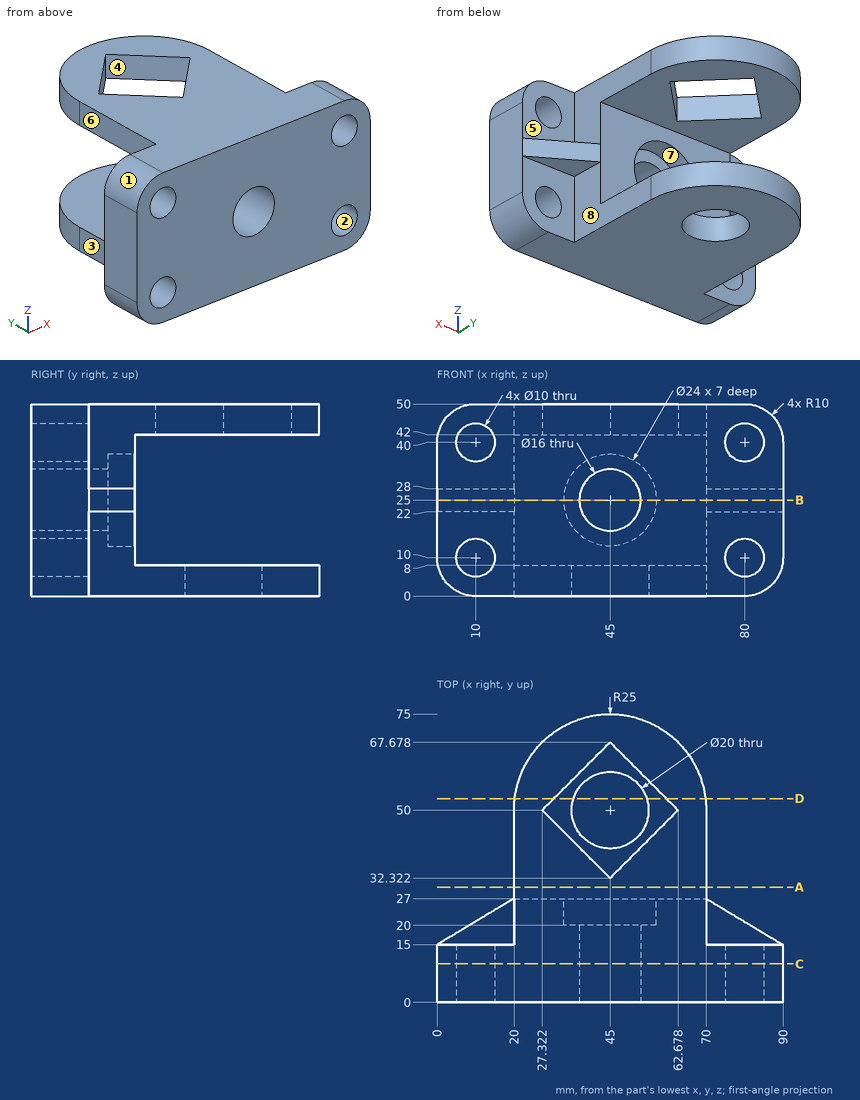
For this review, use the dimensioned drawing (mm, ordinates from the lowest corner) and the shaded views. A direction names the side the tool comes from. Coordinates: 2 decimals unless noted, no trailing zeros. Order: outer loops, then holes, each group sorted by start corner. A loop starts at its lowest first (then second) coordinate and runs counter-clockwise, first axis right, second up. Notation, with made-up numbers: (41.25, 64) - (73.25, 64) arc R18 cw to (73.25, 85) - close; hole circle Ø7 at (61, 38.25). An arc over 180 degrees is marked (long way). Use one line per item in the form item = value.
Q1. Draft analysis for pull direction Z (two halves, no side actions). For the marked faces 1, 2 and 3, state which applies: +Z half, -Z half, draft (parallel to the pull), parting line (faces both ways), or undercut.
Checked values:
face_1 = +Z half
face_2 = undercut
face_3 = draft
Q2. For probe 1 along X at (y, z) = (4, 40); probe 2 along Z at (x, y) = (8, 9); probe 3 along X at (y, z) = (6.75, 25), list the stretches that pass through material, from the lowest coordinate up. Write a range as from..to.
Checked values:
probe_1 = 0..5, 15..75, 85..90
probe_2 = 0.2..5.42, 14.58..35.42, 44.58..49.8
probe_3 = 0..37, 53..90
Q3. Consider section D-D (y = 53). Give the boundary of the cut face in (x, z).
Checked values:
outline = (20.18, 0) - (35.46, 0) - (35.46, 8) - (20.18, 8) - close; (20.18, 42) - (30.32, 42) - (30.32, 50) - (20.18, 50) - close; (54.54, 0) - (69.82, 0) - (69.82, 8) - (54.54, 8) - close; (59.68, 42) - (69.82, 42) - (69.82, 50) - (59.68, 50) - close
Q4. Consider section B-B (z = 25). Give the boundary of the cut face in (x, y).
Checked values:
outline = (0, 0) - (37, 0) - (37, 20) - (33, 20) - (33, 27) - (20, 27) - (0, 15) - close; (53, 0) - (90, 0) - (90, 15) - (70, 27) - (57, 27) - (57, 20) - (53, 20) - close
Q5. Consider section C-C (y = 10). Give the boundary of the cut face in (x, z).
Checked values:
outline = (0, 10) arc R10 ccw to (10, 0) - (80, 0) arc R10 ccw to (90, 10) - (90, 40) arc R10 ccw to (80, 50) - (10, 50) arc R10 ccw to (0, 40) - close; hole circle Ø10 at (10, 10); hole circle Ø10 at (10, 40); hole circle Ø16 at (45, 25); hole circle Ø10 at (80, 10); hole circle Ø10 at (80, 40)
Q6. For P1, Ø11, axis at y = 29.5, z = 15.5, coming from the +X side; P2, Ø6, axis at x = 76, z = 35, coming from the +Y side; P3, Ø12, axis at y = 37, z = 6.5, coming from the -X side, all flat-tipped, find the tip position at first contact; note any pin that passes through.
Checked values:
P1 = 70
P2 = 15
P3 = 20
Q7. Consider section A-A (y = 30). Give the boundary of the cut face in (x, z), then the cut area to 3 significant figures.
Checked values:
outline = (20, 0) - (70, 0) - (70, 8) - (20, 8) - close; (20, 42) - (70, 42) - (70, 50) - (20, 50) - close
area = 800 mm2
Q8. For the marked faces 4, 5, 6, 7 and 8, list the 3-axis set-ups (+Z, -Z, +X, -X, +Y, -Y) from which the entire face can be reached by the end or side of a thin tool; tool diameter is ignored.
Checked values:
face_4 = +Z
face_5 = +Z, +X, +Y
face_6 = +Z, -X, +Y
face_7 = +Y
face_8 = -Z, +X, +Y
